For this review, take the finished solid that the model builds, in its own axes (mm). Round coordinates to 2 decimals unless told otherwise and drop trailing zeros. Order: outer loops, then holes, each group sorted by start corner. A loop starts at its lowest first (then second) coordinate and runs counter-clockwise, first axis right, second up. Notation, with made-up numbers: (34.5, 67.25) -> (51.5, 67.25) arc R21 cw to (51.5, 76.25) -> close; hole circle Ø3 at (65, 46). An arc over 180 degrees is marked (long way). Answer in a Markdown table with one row per item.
```python
from build123d import *

# Parameters (mm, degrees)
SKETCH2_R   = 5
SKETCH2_R_2 = 4


with BuildPart() as part:
    # Sweep1: sweep along a path in Sketch1
    with BuildLine(Plane.XY) as sweep1_path:
        Line((0, 0), (10, 0))
        ThreePointArc((10, 0), (17.071067812, -2.928932188), (20, -10))
        Line((20, -10), (20, -30))
    # Sketch2 → Sweep1 (sweep)
    with BuildSketch(Plane(origin=(0, 0, 0), x_dir=(0, 0, -1), z_dir=(1, 0, 0))):
        Circle(SKETCH2_R)
        Circle(SKETCH2_R_2, mode=Mode.SUBTRACT)
    sweep(path=sweep1_path.line)


solid = part.part
```
Q1. Take a section at A-A, the plane z = 0. Write out the cut boundary in (x, y), then the cut area to 3 significant figures.
Answer key:
| item | result |
|---|---|
| outline | (0, -5) -> (10, -5) arc R5 cw to (15, -10) -> (15, -30) -> (16, -30) -> (16, -10) arc R6 ccw to (10, -4) -> (0, -4) -> close; (0, 4) -> (10, 4) arc R14 cw to (24, -10) -> (24, -30) -> (25, -30) -> (25, -10) arc R15 ccw to (10, 5) -> (0, 5) -> close |
| area | 91.4 mm^2 |
Q2. To check wall thickness, follow probe 1 along Y at (x, z) = (3.25, 0); probe 2 along X at (y, z) = (-11.5, 1). State the ranges of each line that lie inside material, in increasing order.
Answer key:
| item | result |
|---|---|
| probe 1 | y = -5 to -4, 4 to 5 |
| probe 2 | x = 15.1 to 16.13, 23.87 to 24.9 |
Q3. Take a section at C-C, the plane x = 1.5. Write out the cut boundary in (y, z).
Answer key:
| item | result |
|---|---|
| outline | circle Ø10 at (0, 0); hole circle Ø8 at (0, 0) |
Q4. Take a section at D-D, the plane z = 2. Write out the cut boundary in (x, y), then the cut area to 3 significant figures.
Answer key:
| item | result |
|---|---|
| outline | (0, -4.58) -> (10, -4.58) arc R5.42 cw to (15.42, -10) -> (15.42, -30) -> (16.54, -30) -> (16.54, -10) arc R6.54 ccw to (10, -3.46) -> (0, -3.46) -> close; (0, 3.46) -> (10, 3.46) arc R13.46 cw to (23.46, -10) -> (23.46, -30) -> (24.58, -30) -> (24.58, -10) arc R14.58 ccw to (10, 4.58) -> (0, 4.58) -> close |
| area | 102 mm^2 |
Q5. Take a section at B-B, the plane y = -17. Write out the cut boundary in (x, z), then the cut area to 3 significant figures.
Answer key:
| item | result |
|---|---|
| outline | circle Ø10 at (20, 0); hole circle Ø8 at (20, 0) |
| area | 28.3 mm^2 |
Q6. The part is to be moulded in two halves that separate along Z. For faces 1 (the face through (5.07, -4.88, 1.08)), 2 (the face through (23.966, -20.14, 0.521)), 3 (the face through (5.07, -3.905, 0.867)), say which applies: +Z half, -Z half, draft (parallel to the pull), parting line (faces both ways), or undercut.
Answer key:
| item | result |
|---|---|
| face 1 | parting line |
| face 2 | undercut |
| face 3 | undercut |
Q7. Clearance check with flat-ended pins moving along their axes: pin 1 Ø1 at (x, y) = (19, -14) entering from -Z; pin 2 Ø1 at (y, z) = (-24, 1.5) entering from +X; pin 3 Ø4 at (y, z) = (-17.5, 3.5) entering from -X. State where each tip first meets the part, or that it passes through.
Answer key:
| item | result |
|---|---|
| pin 1 | stops at z = -4.97 |
| pin 2 | stops at x = 24.9 |
| pin 3 | stops at x = 15.23 |
